from build123d import *

# Parameters (mm, degrees)
SKETCH_1_W             = 250
SKETCH_1_H             = 280
SKETCH_1_R             = 43
SKETCH_1_R_2           = 35
EXTRUDE_1_DEPTH        = 20
HOLE_WIZARD_M8_1_D     = 6.8
HOLE_WIZARD_M6_1_D     = 5
SKETCH_6_R             = 111
CUT_EXTRUDE_1_DEPTH    = 4
CHAMFER_1_SIZE         = 10
HOLE_WIZARD_M6_2_D     = 5
HOLE_WIZARD_M6_3_D     = 5
HOLE_WIZARD_M6_3_DEPTH = 15
HOLE_WIZARD_M6_3_TIP   = 1.502151548


with BuildPart() as part:
    # 草图1 → 凸台-拉伸1 (new body)
    with BuildSketch(Plane.XY):
        Rectangle(SKETCH_1_W, SKETCH_1_H)
        with Locations((0, -14)):
            Circle(SKETCH_1_R, mode=Mode.SUBTRACT)
        with Locations((0, 88.5)):
            Circle(SKETCH_1_R_2, mode=Mode.SUBTRACT)
    extrude(amount=EXTRUDE_1_DEPTH)

    # M8 螺纹孔1 (through all)
    with Locations(Plane.XY.offset(20)):
        with Locations((-39.799076966, 82.083471381), (39.799076966, 82.083471381), (96.083471381, 25.799076966), (96.083471381, -53.799076966), (39.799076966, -110.083471381), (-39.799076966, -110.083471381), (-96.083471381, -53.799076966), (-96.083471381, 25.799076966)):
            Hole(HOLE_WIZARD_M8_1_D / 2)

    # M6 螺纹孔1 (through all)
    with Locations(Plane(origin=(0, 0, 0), x_dir=(-1, 0, 0), z_dir=(0, 0, -1))):
        with Locations((0, 88.5), (32, 120.5), (-32, 56.5), (-32, 120.5), (32, 56.5)):
            Hole(HOLE_WIZARD_M6_1_D / 2)

    # 草图6 → 切除-拉伸1 (cut)
    with BuildSketch(Plane(origin=(0, 0, 0), x_dir=(-1, 0, 0), z_dir=(0, 0, -1))):
        with Locations((0, -14)):
            Circle(SKETCH_6_R)
    extrude(amount=-CUT_EXTRUDE_1_DEPTH, mode=Mode.SUBTRACT)

    # 倒角1
    chamfer_1_edges = [part.edges().sort_by_distance(p)[0] for p in [
        (125, -140, 10),
        (-125, -140, 10),
        (-125, 140, 10),
        (125, 140, 10),
    ]]
    chamfer(chamfer_1_edges, length=CHAMFER_1_SIZE)

    # M6 螺纹孔2 (through all)
    with Locations(Plane(origin=(0, 0, 0), x_dir=(-1, 0, 0), z_dir=(0, 0, -1))):
        with Locations((103, 125), (-103, 125)):
            Hole(HOLE_WIZARD_M6_2_D / 2)

    # M6 螺纹孔3
    with Locations(Plane(origin=(0, 140, 0), x_dir=(1, 0, 0), z_dir=(0, 1, 0))):
        with Locations((0, -10)):
            Hole(HOLE_WIZARD_M6_3_D / 2, depth=HOLE_WIZARD_M6_3_DEPTH)
            with Locations((0, 0, -(HOLE_WIZARD_M6_3_DEPTH + HOLE_WIZARD_M6_3_TIP / 2))):  # 118° drill point
                Cone(0, HOLE_WIZARD_M6_3_D / 2, HOLE_WIZARD_M6_3_TIP, mode=Mode.SUBTRACT)


solid = part.part
Design review of the part built by this model. Coordinates are the model's own, in mm. A direction names the side the tool comes from. Give positions to 0.01 mm unless a question says otherwise; leave off trailing zeros. Loops run counter-clockwise (first coordinate to the right, second up) from the corner with the lowest first, then second, coordinate; pieces in that order, holes last. Notation, with made-up numbers: M 74.5,2 L 91.5,2 A28 cw 91.5,30 Z; hole C 25,-21.5 d2. An arc over 180 degrees is marked long. Write item = value, one per line.
Q1. Insertion check: pin 1 (4 mm diameter, centred on x = -39.8, y = 82.08, fed in from -Z); pin 2 (5 mm diameter, centred on x = 39, y = 85.5, fed in from -Z). Each pin has a flat end and moves straight along its axis. Give the tip position at first contact, or say it passes through.
Output values:
pin_1 = through
pin_2 = 4
Q2. We need section A-A (y = -14). Give the boundary of the cut face in (x, z).
Output values:
outline = M -125,0 L -111,0 L -111,4 L -43,4 L -43,20 L -125,20 Z; M 43,4 L 111,4 L 111,0 L 125,0 L 125,20 L 43,20 Z
Q3. We need section C-C (y = 71). Give the boundary of the cut face in (x, z).
Output values:
outline = M -125,0 L -71.39,0 L -71.39,4 L -30.31,4 L -30.31,20 L -125,20 Z; M 30.31,4 L 71.39,4 L 71.39,0 L 125,0 L 125,20 L 30.31,20 Z
Q4. To check wall thickness, follow line 1 (Y direction, x = 0, z = 16.75); line 2 (Y direction, x = -96, z = 11.75); line 3 (X direction, y = 24, z = 10.75). State the ranges of each line that lie inside material, in increasing order. Write a range as [from, to].
Output values:
line_1 = [-140, -57], [29, 53.5], [123.5, 140]
line_2 = [-140, -57.2], [-50.4, 22.4], [29.2, 140]
line_3 = [-125, -98.97], [-93.2, -20.12], [20.12, 93.2], [98.97, 125]
Q5. For faces 4 (the cylindrical face through (98.78, 23.73, 11.89)), 5 (the cylindrical face through (4.384, -124.913, 1.972)), list the 3-axis set-ups (+Z, -Z, +X, -X, +Y, -Y) from which the entire face can be reached by the end or side of a thin tool; tool diameter is ignored.
Output values:
face_4 = +Z, -Z
face_5 = -Z
Q6. We need section D-D (x = -61). Give the boundary of the cut face in (y, z), plus the area to 3 significant figures.
Output values:
outline = M -140,0 L -106.74,0 L -106.74,4 L 78.74,4 L 78.74,0 L 140,0 L 140,20 L -140,20 Z
area = 4,860 mm^2
Q7. Draft analysis for pull direction Y (two halves, no side actions). For faces 1 (the flat face through (-2, -140, 10)), 2 (the flat face through (2, -63, 4)), 3 (the flat face through (-125, -2, 10)), state which applies: +Y half, -Y half, draft (parallel to the pull), parting line (faces both ways), or undercut.
Output values:
face_1 = -Y half
face_2 = undercut
face_3 = draft
Q8. We need section B-B (x = -14.5). Give the boundary of the cut face in (y, z), plus the area to 3 significant figures.
Output values:
outline = M -140,0 L -124.05,0 L -124.05,4 L -54.48,4 L -54.48,20 L -140,20 Z; M 26.48,4 L 56.64,4 L 56.64,20 L 26.48,20 Z; M 120.36,0 L 140,0 L 140,20 L 120.36,20 Z
area = 2,310 mm^2
